from build123d import *

# Parameters (mm, degrees)
SKETCH1_R           = 1.5
BOSS_EXTRUDE1_DEPTH = 2


with BuildPart() as part:
    # Sketch1 → Boss-Extrude1 (new body)
    with BuildSketch(Plane(origin=(0, 0, 0), x_dir=(1, 0, 0), z_dir=(0, 1, 0))):
        with BuildLine():
            Line((-13, -2.5), (13, -2.5))
            ThreePointArc((13, -2.5), (14.414213562, -1.914213562), (15, -0.5))
            Line((15, -0.5), (15, 0.5))
            ThreePointArc((15, 0.5), (14.414213562, 1.914213562), (13, 2.5))
            Line((13, 2.5), (-13, 2.5))
            ThreePointArc((-13, 2.5), (-14.414213562, 1.914213562), (-15, 0.5))
            Line((-15, 0.5), (-15, -0.5))
            ThreePointArc((-15, -0.5), (-14.414213562, -1.914213562), (-13, -2.5))
        make_face()
        with Locations(Location((12, 0, 0), (0, 0, 270))):
            Circle(SKETCH1_R, mode=Mode.SUBTRACT)
        with Locations(Location((-12, 0, 0), (0, 0, 270))):
            Circle(SKETCH1_R, mode=Mode.SUBTRACT)
    extrude(amount=BOSS_EXTRUDE1_DEPTH)


solid = part.part
Build history of the part. All positions in model axes, mm. Round coordinates to 2 decimals unless told otherwise and drop trailing zeros. Write each loop counter-clockwise with the first axis right and the second up, starting at its lowest first coordinate (ties: lowest second). Pieces come first, ordered by that corner, then holes. Notation, with made-up numbers: (59.25, -6.5) - (66.25, -6.5) arc R10 ccw to (66.25, -0.5) - close; hole circle Ø6 at (80.5, 37.5). An arc over 180 degrees is marked (long way). Use CSV: the item, a comma, the result in double quotes.
(1) Mould opens along X. For faces 1 (the flat face through (0, 1, 2.5)), 2 (the cylindrical face through (-11.55, 0.99, 1.43)), 3 (the flat face through (-15, 1, 0)) say: pulls with the +X half, pulls with the -X half, needs draft (parallel to the pull), parting line crosses it, or undercut.
Response:
face 1,"needs draft"
face 2,"undercut"
face 3,"pulls with the -X half"
(2) Band-saw the part on C-C (y = 0.55). Write the cut outline in (x, z).
Response:
outline,"(-15, -0.5) arc R2 ccw to (-13, -2.5) - (13, -2.5) arc R2 ccw to (15, -0.5) - (15, 0.5) arc R2 ccw to (13, 2.5) - (-13, 2.5) arc R2 ccw to (-15, 0.5) - close; hole circle Ø3 at (-12, 0); hole circle Ø3 at (12, 0)"
(3) Band-saw the part on A-A (z = 0). Write the cut outline in (x, y), plus the area to 3 significant figures.
Response:
outline,"(-15, 0) - (-13.5, 0) - (-13.5, 2) - (-15, 2) - close; (-10.5, 0) - (10.5, 0) - (10.5, 2) - (-10.5, 2) - close; (13.5, 0) - (15, 0) - (15, 2) - (13.5, 2) - close"
area,"48.0 mm²"
(4) Band-saw the part on D-D (x = -11.25). Write the cut outline in (y, z), plus the area to 3 significant figures.
Response:
outline,"(0, -2.5) - (2, -2.5) - (2, -1.3) - (0, -1.3) - close; (0, 1.3) - (2, 1.3) - (2, 2.5) - (0, 2.5) - close"
area,"4.80 mm²"
(5) Wall check: line 1 (X direction, y = 0.6, z = 0); line 2 (X direction, y = 0.4, z = -0.9); line 3 (X direction, y = 1.3, z = -2.3). Give the ranges that are in metal, low to high.
Response:
line 1,"-15 to -13.5, -10.5 to 10.5, 13.5 to 15"
line 2,"-14.96 to -13.2, -10.8 to 10.8, 13.2 to 14.96"
line 3,"-13.87 to 13.87"
(6) Band-saw the part on B-B (x = 12). Write the cut outline in (y, z), plus the area to 3 significant figures.
Response:
outline,"(0, -2.5) - (2, -2.5) - (2, -1.5) - (0, -1.5) - close; (0, 1.5) - (2, 1.5) - (2, 2.5) - (0, 2.5) - close"
area,"4.00 mm²"
